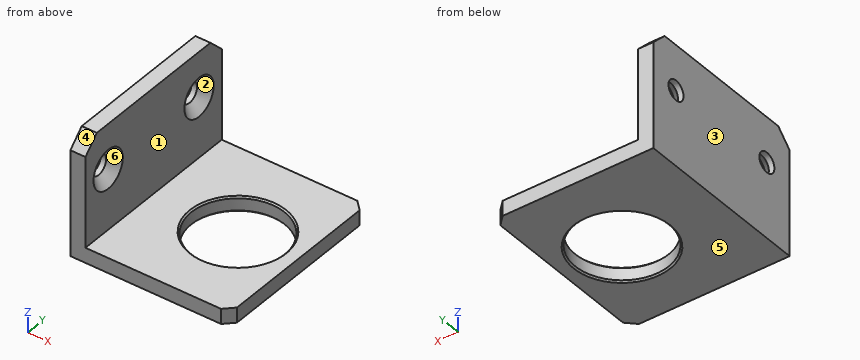
from build123d import *

# Parameters (mm, degrees)
EXTRUDE_1_DEPTH          = 60
SKETCH_2_R               = 15.5
CUT_EXTRUDE_1_DEPTH      = 90.493016487
CHAMFER_1_SIZE           = 3
CHAMFER_2_SIZE           = 5
HOLE_WIZARD_1_AT_2_COUNT = 2
HOLE_WIZARD_1_AT_2_PITCH = 40
CHAMFER_3_SIZE           = 0.5


with BuildPart() as part:
    # 草图1 → 凸台-拉伸1 (new body)
    with BuildSketch(Plane(origin=(0, 0, 0), x_dir=(1, 0, 0), z_dir=(0, 1, 0))):
        Polygon((0, 0), (0, 40), (53, 40), (53, 35), (5, 35), (5, 0), align=None)
    extrude(amount=EXTRUDE_1_DEPTH)

    # 草图2 → 切除-拉伸1 (cut, through all)
    with BuildSketch(Plane(origin=(0, 0, -40), x_dir=(-1, 0, 0), z_dir=(0, 0, -1))):
        with Locations((-33, 30)):
            Circle(SKETCH_2_R)
    extrude(amount=-CUT_EXTRUDE_1_DEPTH, mode=Mode.SUBTRACT)

    # 倒角1
    chamfer_1_edges = [part.edges().sort_by_distance(p)[0] for p in [
        (53, 60, -37.5),
        (53, 0, -37.5),
    ]]
    chamfer(chamfer_1_edges, length=CHAMFER_1_SIZE)

    # 倒角2
    chamfer_2_edges = [part.edges().sort_by_distance(p)[0] for p in [
        (2.5, 60, 0),
        (2.5, 0, 0),
    ]]
    chamfer(chamfer_2_edges, length=CHAMFER_2_SIZE)

    # 草图3 → 打孔尺寸根据十字槽沉头木螺钉的类型1 (revolve, cut)
    with BuildSketch(Plane(origin=(5, 10, -15), x_dir=(0, 0, -1), z_dir=(0, 1, 0))):
        Polygon((0, 0), (0, 5), (3.3, 5), (3.3, 3.15), (6.45, 0), align=None)
    hole_wizard_1 = revolve(axis=Axis((11.35, 10, -15), (-1, 0, 0)), mode=Mode.SUBTRACT)

    # 打孔尺寸根据十字槽沉头木螺钉的类型1 at 2: 打孔尺寸根据十字槽沉头木螺钉的类型1 ×2
    with Locations(*[(0, i * HOLE_WIZARD_1_AT_2_PITCH, 0) for i in range(1, HOLE_WIZARD_1_AT_2_COUNT)]):
        add(hole_wizard_1, mode=Mode.SUBTRACT)

    # 倒角3
    chamfer_3_edges = [part.edges().sort_by_distance(p)[0] for p in [
        (48.5, 30, -35),
        (48.5, 30, -40),
    ]]
    chamfer(chamfer_3_edges, length=CHAMFER_3_SIZE)


solid = part.part
Geometry check sheet. Reference: the model listing, model coordinates, mm. Face numbers are marked on the shaded views. A direction names the side the tool comes from. Round coordinates to 2 decimals unless told otherwise and drop trailing zeros. Order: outer loops, then holes, each group sorted by start corner. A loop starts at its lowest first (then second) coordinate and runs counter-clockwise, first axis right, second up. Notation, with made-up numbers: M 7,6.25 L 48,6.25 A22 cw 48,41.25 Z; hole C 22,40.25 d9. An arc over 180 degrees is marked long. Answer in a Markdown table with one row per item. Add a question column.
Item 1: Material ranges on L1, parallel to Z at x = 1.35, y = 10; L2, parallel to Y at x = 33, z = -36.35; L3, parallel to Z at x = 29.5, y = 7.5, recorded low to high. Write a range as [from, to].
Item 2: Set-up check for the marked faces 1 and 2: record each of +Z, -Z, +X, -X, +Y, -Y from which the full face is reachable in a straight line by a thin tool's end or side.
Item 3: Sectioned sample at A-A, the plane x = 33. Enter the section's corners in (y, z), plus the area to 4 significant figures.
Item 4: Sectioned sample at D-D, the plane y = 30. Enter the section's corners in (x, z).
Item 5: Depth check by flat-ended pin: pin 1 Ø8 at (y, z) = (46.5, -5) entering from +X. Enter the tip coordinate at first touch or a pass-through.
Item 6: Sectioned sample at B-B, the plane y = 50. Enter the section's corners in (x, z), plus the area to 3 significant figures.
Item 7: Draft check along Z on the marked faces 3, 4, 5 and 6. Enter one of: released by +Z, released by -Z, zero draft, split by the parting line, or undercut.
Item 8: Sectioned sample at C-C, the plane z = -15. Enter the section's corners in (x, y), plus the area to 3 significant figures.
Filled in:
| question | item | result |
|---|---|---|
| 1 | L1 | z = [-40, -18.3], [-11.7, 0] |
| 1 | L2 | y = [0, 14.5], [45.5, 60] |
| 1 | L3 | z = [-40, -35] |
| 2 | face 1 | +Z, +X, +Y, -Y |
| 2 | face 2 | +X |
| 3 | outline | M 0,-40 L 14,-40 L 14.5,-39.5 L 14.5,-35.5 L 14,-35 L 0,-35 Z; M 45.5,-39.5 L 46,-40 L 60,-40 L 60,-35 L 46,-35 L 45.5,-35.5 Z |
| 3 | area | 144.5 mm² |
| 4 | outline | M 0,-40 L 17,-40 L 17.5,-39.5 L 17.5,-35.5 L 17,-35 L 5,-35 L 5,0 L 0,0 Z; M 48.5,-39.5 L 49,-40 L 53,-40 L 53,-35 L 49,-35 L 48.5,-35.5 Z |
| 5 | pin 1 | stops at x = 5 |
| 6 | outline | M 0,-40 L 53,-40 L 53,-35 L 5,-35 L 5,-21.45 L 1.85,-18.3 L 0,-18.3 Z; M 0,-11.7 L 1.85,-11.7 L 5,-8.55 L 5,0 L 0,0 Z |
| 6 | area | 397 mm² |
| 7 | face 3 | zero draft |
| 7 | face 4 | released by +Z |
| 7 | face 5 | released by -Z |
| 7 | face 6 | undercut |
| 8 | outline | M 0,0 L 5,0 L 5,3.55 L 1.85,6.7 L 0,6.7 Z; M 0,13.3 L 1.85,13.3 L 5,16.45 L 5,43.55 L 1.85,46.7 L 0,46.7 Z; M 0,53.3 L 1.85,53.3 L 5,56.45 L 5,60 L 0,60 Z |
| 8 | area | 214 mm² |
